from build123d import *

# Parameters (mm, degrees)
EXTRUDE_1_DEPTH = 2
CHAMFER_1_SIZE  = 3


with BuildPart() as part:
    # 草图1 → 凸台-拉伸1 (new body)
    with BuildSketch(Plane.XY):
        Polygon((0, 0), (43.5, 0), (43.5, -32), (10, -60), (0, -60), align=None)
    extrude(amount=EXTRUDE_1_DEPTH)

    # 倒角1
    chamfer_1_edges = [part.edges().sort_by_distance(p)[0] for p in [
        (0, 0, 1),
        (43.5, 0, 1),
    ]]
    chamfer(chamfer_1_edges, length=CHAMFER_1_SIZE)


solid = part.part
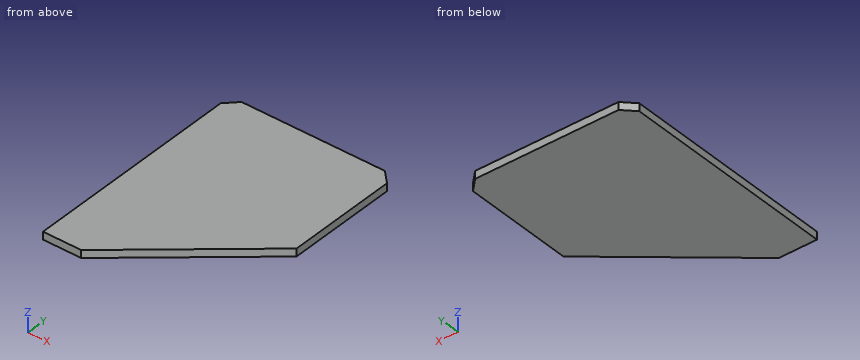
CAD build for the part. Positions are in the model's coordinates, mm. Round coordinates to 2 decimals unless told otherwise and drop trailing zeros. Order: outer loops, then holes, each group sorted by start corner. A loop starts at its lowest first (then second) coordinate and runs counter-clockwise, first axis right, second up. Notation, with made-up numbers: (-15, 80) -> (-3, 80) arc R30 ccw to (-3, 117) -> close; hole circle Ø11 at (13.5, 31.25). An arc over 180 degrees is marked (long way). Write item = value, one per line. Start each with the question number.
(1) Probe line 1 (X direction, y = -52, z = 0.15); line 2 (Y direction, x = 16.5, z = 0.7); line 3 (X direction, y = -37, z = 1.65). List the from-to ranges inside material, lowest first. Write a range as [from, to].
(2) Cut at B-B, the plane x = 24.5. List the corners of the cut face in (y, z).
(3) Cut at C-C, the plane y = -43. List the corners of the cut face in (x, z).
(4) Cut at A-A, the plane z = 1.5. List the corners of the cut face in (x, y), then the cut area to 3 significant figures.
Model answer:
q1.line_1 = [0, 19.57]
q1.line_2 = [-54.57, 0]
q1.line_3 = [0, 37.52]
q2.outline = (-47.88, 0) -> (0, 0) -> (0, 2) -> (-47.88, 2) -> close
q3.outline = (0, 0) -> (30.34, 0) -> (30.34, 2) -> (0, 2) -> close
q4.outline = (0, -60) -> (10, -60) -> (43.5, -32) -> (43.5, -3) -> (40.5, 0) -> (3, 0) -> (0, -3) -> close
q4.area = 2,130 mm2
